The model under review builds one solid part; all positions refer to its coordinate system, in mm. A direction names the side the tool comes from. Give positions to 0.01 mm unless a question says otherwise; leave off trailing zeros. Write each loop counter-clockwise with the first axis right and the second up, starting at its lowest first coordinate (ties: lowest second). Pieces come first, ordered by that corner, then holes. Notation, with made-up numbers: (60.5, -20.75) - (110.5, -20.75) arc R21 ccw to (110.5, -7.75) - close; hole circle Ø9 at (6, -34.75). An arc over 180 degrees is marked (long way). Write item = value, one per line.
```python
from build123d import *

# Parameters (mm, degrees)
BASE_BLOCK_108X50X28_DEPTH     = 28
JAW_SLOT_PROFILE_W             = 22
JAW_SLOT_PROFILE_H             = 6
JAW_SLOT_CUT_DEPTH             = 40
BORE_28_PROFILE_R              = 14
BORE_28_DEPTH                  = 66.76473219
THROUGH_SLOT_CUT_DEPTH         = 53
SIDE_GROOVE_PROFILE_W          = 22
SIDE_GROOVE_PROFILE_H          = 8
SIDE_GROOVE_CUT_DEPTH          = 40
END_CHAMFER_11X45_SIZE         = 11
ARC_RECESS_6_DEEP_DEPTH        = 6
ARC_POCKET_AND_HOLES_PROFILE_R = 5
ARC_POCKET_AND_HOLES_CUT_DEPTH = 66.76473219


with BuildPart() as part:
    # Base Block Profile → Base Block 108x50x28 (new body)
    with BuildSketch(Plane(origin=(0, 0, 0), x_dir=(1, 0, 0), z_dir=(0, 1, 0))):
        Polygon((-54, 25), (43, 25), (54, 25), (54, -25), (43, -25), (-54, -25), align=None)
    extrude(amount=BASE_BLOCK_108X50X28_DEPTH)

    # Jaw Slot Profile → Jaw Slot Cut (cut)
    with BuildSketch(Plane(origin=(54, 0, 0), x_dir=(0, 0, -1), z_dir=(1, 0, 0))):
        with Locations((0, 25)):
            Rectangle(JAW_SLOT_PROFILE_W, JAW_SLOT_PROFILE_H)
    extrude(amount=-JAW_SLOT_CUT_DEPTH, mode=Mode.SUBTRACT)

    # Bore Ø28 Profile → Bore Ø28 (cut, through all)
    with BuildSketch(Plane(origin=(0, 28, 0), x_dir=(1, 0, 0), z_dir=(0, 1, 0))):
        with Locations(Location((14, 0, 0), (0, 0, 270))):
            Circle(BORE_28_PROFILE_R)
    extrude(amount=-BORE_28_DEPTH, mode=Mode.SUBTRACT)

    # Through Slot Profile → Through Slot Cut (cut)
    with BuildSketch(Plane(origin=(54, 0, 0), x_dir=(0, 0, -1), z_dir=(1, 0, 0))):
        Polygon((-25, 28), (-11, 28), (25, 28), (25, 22), (-11, 22), (-25, 22), align=None)
    extrude(amount=-THROUGH_SLOT_CUT_DEPTH, mode=Mode.SUBTRACT)

    # Side Groove Profile → Side Groove Cut (cut)
    with BuildSketch(Plane(origin=(54, 0, 0), x_dir=(0, 0, -1), z_dir=(1, 0, 0))):
        with Locations((0, 18)):
            Rectangle(SIDE_GROOVE_PROFILE_W, SIDE_GROOVE_PROFILE_H)
    extrude(amount=-SIDE_GROOVE_CUT_DEPTH, mode=Mode.SUBTRACT)

    # End Chamfer 11x45°
    end_chamfer_11x45_edges = [part.edges().sort_by_distance(p)[0] for p in [
        (54, 11, 25),
        (54, 11, -25),
    ]]
    chamfer(end_chamfer_11x45_edges, length=END_CHAMFER_11X45_SIZE)

    # Arc Recess Profile → Arc Recess 6 Deep (cut)
    with BuildSketch(Plane(origin=(0, 28, 0), x_dir=(1, 0, 0), z_dir=(0, 1, 0))):
        with BuildLine():
            Line((-40.543560573, -25), (-17.224989992, -25))
            ThreePointArc((-17.224989992, -25), (-26, 0), (-17.224989992, 25))
            Line((-17.224989992, 25), (-40.543560573, 25))
            ThreePointArc((-40.543560573, 25), (-46, 0), (-40.543560573, -25))
        make_face()
    extrude(amount=-ARC_RECESS_6_DEEP_DEPTH, mode=Mode.SUBTRACT)

    # Arc Pocket and Holes Profile → Arc Pocket and Holes Cut (cut, through all)
    with BuildSketch(Plane(origin=(0, 28, 0), x_dir=(1, 0, 0), z_dir=(0, 1, 0))):
        with Locations(Location((-35.385362758, 11.497401318, 0), (0, 0, 270))):
            Circle(ARC_POCKET_AND_HOLES_PROFILE_R)
        with Locations(Location((-35.385362758, -11.497401318, 0), (0, 0, 270))):
            Circle(ARC_POCKET_AND_HOLES_PROFILE_R)
    extrude(amount=-ARC_POCKET_AND_HOLES_CUT_DEPTH, mode=Mode.SUBTRACT)


solid = part.part
```
1. Draft analysis for pull direction Z (two halves, no side actions). For faces 6 (the flat face through (-5, 11, -25)), 7 (the flat face through (-35, 22, 0)), 8 (the flat face through (39, 18, -11)), 9 (the flat face through (1, 25, -15)), state which applies: +Z half, -Z half, draft (parallel to the pull), parting line (faces both ways), or undercut.
Findings below:
face_6 = -Z half
face_7 = undercut
face_8 = undercut
face_9 = draft
2. Machinability: for faces 1 (the flat face through (-49, 28, 0)), 2 (the cylindrical face through (-26, 25, 0)), 3 (the flat face through (28, 22, 17)), 4 (the cylindrical face through (-30.43, 11.15, -12.15)), 5 (the flat face through (39, 18, 11)), which of the approach directions +Z, -Z, +X, -X, +Y, -Y give a long, thin tool a straight path to every point of the face, cutting with its end or side? Answer none if there is none.
Findings below:
face_1 = +Z, -Z, +X, -X, +Y
face_2 = +Y
face_3 = +Z, -Z, +X, +Y
face_4 = +Y, -Y
face_5 = +X, +Y
3. Insertion check: P1, Ø6.5, axis at x = 31.5, z = -2, coming from the +Y side; P2, Ø22, axis at x = 20.5, z = 17, coming from the +Y side; P3, Ø1.8, axis at y = 26.5, z = -10, coming from the +X side. Each pin has a flat end and moves straight along its axis. Give the tip position at first contact, or say it passes through.
Findings below:
P1 = 14
P2 = 22
P3 = 1
4. Take a section at D-D on z = -15. Give the boundary of the cut face in (x, y), and give its area (3 significant figures).
Findings below:
outline = (-54, 0) - (-38.95, 0) - (-38.95, 22) - (-44.09, 22) - (-44.09, 28) - (-54, 28) - close; (-31.82, 0) - (53, 0) - (53, 22) - (1, 22) - (1, 28) - (-23.08, 28) - (-23.08, 22) - (-31.82, 22) - close
area = 2,400 mm²
5. For line 1 (Z direction, x = 14, y = 12.25); line 2 (Y direction, x = 37, z = 13.5); line 3 (Z direction, x = 41.5, y = 21.5), list the stretches that pass through material, from the lowest coordinate up. Write a range as from..to.
Findings below:
line_1 = -25..-14, 14..25
line_2 = 0..22
line_3 = -25..-11, 11..25
6. Take a section at C-C on y = 17. Give the boundary of the cut face in (x, z).
Findings below:
outline = (-54, -25) - (43, -25) - (54, -14) - (54, -11) - (22.66, -11) arc R14 cw (long way) to (22.66, 11) - (54, 11) - (54, 14) - (43, 25) - (-54, 25) - close; hole circle Ø10 at (-35.39, -11.5); hole circle Ø10 at (-35.39, 11.5)
7. Take a section at B-B on x = 14. Give the boundary of the cut face in (y, z), and give its area (3 significant figures).
Findings below:
outline = (0, -25) - (22, -25) - (22, -14) - (0, -14) - close; (0, 14) - (22, 14) - (22, 25) - (0, 25) - close
area = 484 mm²
8. Take a section at A-A on z = 0. Give the boundary of the cut face in (x, y).
Findings below:
outline = (-54, 0) - (0, 0) - (0, 28) - (-26, 28) - (-26, 22) - (-46, 22) - (-46, 28) - (-54, 28) - close; (28, 0) - (54, 0) - (54, 14) - (28, 14) - close
